Build history of the part. All positions in model axes, mm. A direction names the side the tool comes from. Round coordinates to 2 decimals unless told otherwise and drop trailing zeros. Loops run counter-clockwise (first coordinate to the right, second up) from the corner with the lowest first, then second, coordinate; pieces in that order, holes last. Notation, with made-up numbers: M 58.5,-35.5 L 74.5,-35.5 A19 cw 74.5,-19.5 Z; hole C 8.25,66.25 d6. An arc over 180 degrees is marked long. Use one line per item in the form item = value. Start each with the question number.
```python
from build123d import *
from OCP.BRepFilletAPI import BRepFilletAPI_MakeChamfer

# Parameters (mm, degrees)
SKETCH1_W           = 180
SKETCH1_H           = 70
BOSS_EXTRUDE1_DEPTH = 10
CUT_EXTRUDE1_DEPTH  = 98.082439195
SKETCH3_R           = 2.5
CUT_EXTRUDE2_DEPTH  = 98.082439195
CHAMFER1_SIZE       = 1
CHAMFER1_SIZE2      = 2.732050808
SKETCH4_R           = 2.55
CUT_EXTRUDE3_DEPTH  = 98.082439195


with BuildPart() as part:
    # Sketch1 → Boss-Extrude1 (new body)
    with BuildSketch(Plane.XY):
        Rectangle(SKETCH1_W, SKETCH1_H)
    extrude(amount=BOSS_EXTRUDE1_DEPTH)

    # Sketch2 → Cut-Extrude1 (cut, through all)
    with BuildSketch(Plane.XY.offset(10)):
        Polygon((-72, 35), (-66.226497308, 25), (-17.773502692, 25), (-12, 35), align=None)
        Polygon((72, 35), (12, 35), (17.773502692, 25), (66.226497308, 25), align=None)
        Polygon((72, -35), (66.226497308, -25), (17.773502692, -25), (12, -35), align=None)
        Polygon((-72, -35), (-12, -35), (-17.773502692, -25), (-66.226497308, -25), align=None)
    extrude(amount=-CUT_EXTRUDE1_DEPTH, mode=Mode.SUBTRACT)

    # Sketch3 → Cut-Extrude2 (cut, through all)
    with BuildSketch(Plane.XY.offset(10)):
        with Locations((-82, 27)):
            Circle(SKETCH3_R)
        with Locations(Location((82, 27, 0), (0, 0, 180))):
            Circle(SKETCH3_R)
        with Locations((82, -27)):
            Circle(SKETCH3_R)
        with Locations(Location((-82, -27, 0), (0, 0, 180))):
            Circle(SKETCH3_R)
    extrude(amount=-CUT_EXTRUDE2_DEPTH, mode=Mode.SUBTRACT)

    # Chamfer1: one chamfer whose edges measure the first distance from different faces: ONE call of the kernel's chamfer builder (chamfer() names one face for all edges)
    chamfer1_edges_1 = [part.edges().sort_by_distance(p)[0] for p in [
        (-72, -35, 5),
    ]]
    chamfer1_side_1 = [part.faces().sort_by_distance(p)[0] for p in [
        (-69.113248654, -30, 5),
    ]]
    chamfer1_edges_2 = [part.edges().sort_by_distance(p)[0] for p in [
        (-12, -35, 5),
    ]]
    chamfer1_side_2 = [part.faces().sort_by_distance(p)[0] for p in [
        (0, -35, 5),
    ]]
    chamfer1_edges_3 = [part.edges().sort_by_distance(p)[0] for p in [
        (72, -35, 5),
    ]]
    chamfer1_side_3 = [part.faces().sort_by_distance(p)[0] for p in [
        (81, -35, 5),
    ]]
    chamfer1_edges_4 = [part.edges().sort_by_distance(p)[0] for p in [
        (12, -35, 5),
    ]]
    chamfer1_side_4 = [part.faces().sort_by_distance(p)[0] for p in [
        (14.886751346, -30, 5),
    ]]
    chamfer1_edges_5 = [part.edges().sort_by_distance(p)[0] for p in [
        (72, 35, 5),
    ]]
    chamfer1_side_5 = [part.faces().sort_by_distance(p)[0] for p in [
        (69.113248654, 30, 5),
    ]]
    chamfer1_edges_6 = [part.edges().sort_by_distance(p)[0] for p in [
        (12, 35, 5),
    ]]
    chamfer1_side_6 = [part.faces().sort_by_distance(p)[0] for p in [
        (0, 35, 5),
    ]]
    chamfer1_edges_7 = [part.edges().sort_by_distance(p)[0] for p in [
        (-72, 35, 5),
    ]]
    chamfer1_side_7 = [part.faces().sort_by_distance(p)[0] for p in [
        (-81, 35, 5),
    ]]
    chamfer1_edges_8 = [part.edges().sort_by_distance(p)[0] for p in [
        (-12, 35, 5),
    ]]
    chamfer1_side_8 = [part.faces().sort_by_distance(p)[0] for p in [
        (-14.886751346, 30, 5),
    ]]
    chamfer1_edges_9 = [part.edges().sort_by_distance(p)[0] for p in [
        (90, -35, 5),
        (-90, -35, 5),
        (-90, 35, 5),
        (90, 35, 5),
    ]]
    chamfer1 = BRepFilletAPI_MakeChamfer(part.part.solid().wrapped)
    for e in chamfer1_edges_1:
        chamfer1.Add(CHAMFER1_SIZE, CHAMFER1_SIZE2, e.wrapped, chamfer1_side_1[0].wrapped)  # the first distance lies on this face
    for e in chamfer1_edges_2:
        chamfer1.Add(CHAMFER1_SIZE, CHAMFER1_SIZE2, e.wrapped, chamfer1_side_2[0].wrapped)  # the first distance lies on this face
    for e in chamfer1_edges_3:
        chamfer1.Add(CHAMFER1_SIZE, CHAMFER1_SIZE2, e.wrapped, chamfer1_side_3[0].wrapped)  # the first distance lies on this face
    for e in chamfer1_edges_4:
        chamfer1.Add(CHAMFER1_SIZE, CHAMFER1_SIZE2, e.wrapped, chamfer1_side_4[0].wrapped)  # the first distance lies on this face
    for e in chamfer1_edges_5:
        chamfer1.Add(CHAMFER1_SIZE, CHAMFER1_SIZE2, e.wrapped, chamfer1_side_5[0].wrapped)  # the first distance lies on this face
    for e in chamfer1_edges_6:
        chamfer1.Add(CHAMFER1_SIZE, CHAMFER1_SIZE2, e.wrapped, chamfer1_side_6[0].wrapped)  # the first distance lies on this face
    for e in chamfer1_edges_7:
        chamfer1.Add(CHAMFER1_SIZE, CHAMFER1_SIZE2, e.wrapped, chamfer1_side_7[0].wrapped)  # the first distance lies on this face
    for e in chamfer1_edges_8:
        chamfer1.Add(CHAMFER1_SIZE, CHAMFER1_SIZE2, e.wrapped, chamfer1_side_8[0].wrapped)  # the first distance lies on this face
    for e in chamfer1_edges_9:
        chamfer1.Add(CHAMFER1_SIZE, e.wrapped)
    add(Compound.cast(chamfer1.Shape()), mode=Mode.REPLACE)

    # Sketch4 → Cut-Extrude3 (cut, through all)
    with BuildSketch(Plane.XY.offset(10)):
        with Locations((-35, 12)):
            Circle(SKETCH4_R)
        with Locations((-11, 12)):
            Circle(SKETCH4_R)
        with Locations((13, 12)):
            Circle(SKETCH4_R)
        with Locations((37, 12)):
            Circle(SKETCH4_R)
        with Locations(Location((37, -12, 0), (0, 0, 180))):
            Circle(SKETCH4_R)
        with Locations(Location((13, -12, 0), (0, 0, 180))):
            Circle(SKETCH4_R)
        with Locations(Location((-11, -12, 0), (0, 0, 180))):
            Circle(SKETCH4_R)
        with Locations(Location((-35, -12, 0), (0, 0, 180))):
            Circle(SKETCH4_R)
    extrude(amount=-CUT_EXTRUDE3_DEPTH, mode=Mode.SUBTRACT)


solid = part.part
```
Q1. Saw through at B-B (y = 27). Give the cut face in (x, z).
Q2. Tool access for faces 1 (the face through (-42, 25, 5)), 2 (the face through (-42, -25, 5)), 3 (the face through (81, -35, 5)): list every direction of +Z, -Z, +X, -X, +Y, -Y with a clear straight run to the whole face (end or side of a thin tool).
Q3. Drop a flat-ended pin along its axis: P1, Ø1, axis at x = 40.5, z = 7, coming from the +Y side. Give the stop position or say it passes through.
Q4. Saw through at D-D (y = 12). Give the cut face in (x, z).
Q5. Saw through at C-C (x = 82). Give the cut face in (y, z).
Q6. Pull direction X, two halves, no side cores. Call faces 4 (the face through (90, 0, 5)), 5 (the face through (-79.5, -27.1, 5.1)), 6 (the face through (-1, -35, 5)): pulls with the +X half, pulls with the -X half, needs draft (parallel to the pull), parting line crosses it, or undercut.
Q7. Wall check: probe 1 along Y at (x, z) = (-82, 1.25); probe 2 along X at (y, z) = (-12, 3.75); probe 3 along Y at (x, z) = (-35, 4.25). Give the ranges that are in metal, low to high.
Q8. Saw through at A-A (x = 37). Give the cut face in (y, z), and give its area (3 significant figures).
Filled in:
q1.outline = M -90,0 L -84.5,0 L -84.5,10 L -90,10 Z; M -79.5,0 L -67.38,0 L -67.38,10 L -79.5,10 Z; M -16.62,0 L 16.62,0 L 16.62,10 L -16.62,10 Z; M 67.38,0 L 79.5,0 L 79.5,10 L 67.38,10 Z; M 84.5,0 L 90,0 L 90,10 L 84.5,10 Z
q2.face_1 = +Z, -Z, +Y
q2.face_2 = +Z, -Z, -Y
q2.face_3 = +Z, -Z, +X, -X, -Y
q3.P1 = 25
q4.outline = M -90,0 L -37.55,0 L -37.55,10 L -90,10 Z; M -32.45,0 L -13.55,0 L -13.55,10 L -32.45,10 Z; M -8.45,0 L 10.45,0 L 10.45,10 L -8.45,10 Z; M 15.55,0 L 34.45,0 L 34.45,10 L 15.55,10 Z; M 39.55,0 L 90,0 L 90,10 L 39.55,10 Z
q5.outline = M -35,0 L -29.5,0 L -29.5,10 L -35,10 Z; M -24.5,0 L 24.5,0 L 24.5,10 L -24.5,10 Z; M 29.5,0 L 35,0 L 35,10 L 29.5,10 Z
q6.face_4 = pulls with the +X half
q6.face_5 = undercut
q6.face_6 = needs draft
q7.probe_1 = -35 to -29.5, -24.5 to 24.5, 29.5 to 35
q7.probe_2 = -90 to -37.55, -32.45 to -13.55, -8.45 to 10.45, 15.55 to 34.45, 39.55 to 90
q7.probe_3 = -25 to -14.55, -9.45 to 9.45, 14.55 to 25
q8.outline = M -25,0 L -14.55,0 L -14.55,10 L -25,10 Z; M -9.45,0 L 9.45,0 L 9.45,10 L -9.45,10 Z; M 14.55,0 L 25,0 L 25,10 L 14.55,10 Z
q8.area = 398 mm²
